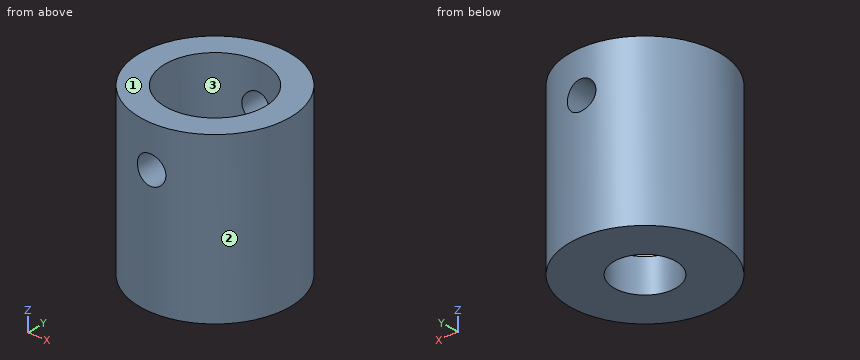
```python
from build123d import *

# Parameters (mm, degrees)
SKETCH1_R               = 58
SKETCH1_R_2             = 24
BOSS_EXTRUDE1_DEPTH     = 128
SKETCH2_R               = 38
CUT_EXTRUDE1_DEPTH      = 102
CUT_EXTRUDE2_DEPTH      = 153.026313512
CUT_EXTRUDE2_DEPTH_BACK = 153.026313512
SKETCH3_R               = 11
SKETCH6_R               = 38.5
CUT_EXTRUDE3_DEPTH      = 68
SKETCH7_R               = 40
CUT_EXTRUDE4_DEPTH      = 4


with BuildPart() as part:
    # Sketch1 → Boss-Extrude1 (new body)
    with BuildSketch(Plane.XY):
        Circle(SKETCH1_R)
        Circle(SKETCH1_R_2, mode=Mode.SUBTRACT)
    extrude(amount=BOSS_EXTRUDE1_DEPTH)

    # Sketch2 → Cut-Extrude1 (cut)
    with BuildSketch(Plane.XY.offset(128)):
        Circle(SKETCH2_R)
    extrude(amount=-CUT_EXTRUDE1_DEPTH, mode=Mode.SUBTRACT)

    # Sketch3 → Cut-Extrude2 (cut, two sides: drawn at the far end of the back side and taken through both)
    with BuildSketch(Plane(origin=(0, 0, 0), x_dir=(1, 0, 0), z_dir=(0, 1, 0)).offset(-CUT_EXTRUDE2_DEPTH_BACK)):
        with Locations(Location((0, -96, 0), (0, 0, 270))):
            Circle(SKETCH3_R)
    extrude(amount=CUT_EXTRUDE2_DEPTH + CUT_EXTRUDE2_DEPTH_BACK, mode=Mode.SUBTRACT)

    # Sketch6 → Cut-Extrude3 (cut)
    with BuildSketch(Plane.XY.offset(128)):
        Circle(SKETCH6_R)
    extrude(amount=-CUT_EXTRUDE3_DEPTH, mode=Mode.SUBTRACT)

    # Sketch7 → Cut-Extrude4 (cut)
    with BuildSketch(Plane.XY.offset(60)):
        Circle(SKETCH7_R)
    extrude(amount=CUT_EXTRUDE4_DEPTH, mode=Mode.SUBTRACT)


solid = part.part
```
For this review, take the finished solid that the model builds, in its own axes (mm). Face numbers are marked on the shaded views. Coordinates: 2 decimals unless noted, no trailing zeros. Loops run counter-clockwise (first coordinate to the right, second up) from the corner with the lowest first, then second, coordinate; pieces in that order, holes last.
1. For line 1 (Z direction, x = 0, y = -50.5); line 2 (Y direction, x = 0, z = 63.1); line 3 (Y direction, x = 0, z = 7), list the stretches that pass through material, from the lowest coordinate up.
2. Mouldability with a two-part tool opening along Y and no side actions: class the marked faces 1, 2 and 3 as +Y half, -Y half, draft (parallel to the pull), parting line (faces both ways), or undercut.
3. Add section A-A, the plane y = 0. Give the boundary of the cut face in (x, z), then the cut area to 3 significant figures.
4. Add section B-B, the plane x = 0. Give the boundary of the cut face in (y, z).
5. Add section C-C, the plane z = 96. Give the boundary of the cut face in (x, y).
6. Insertion check: P1, Ø1.5, axis at x = 30.5, y = 15, coming from the +Z side; P2, Ø10, axis at y = 38.5, z = 41, coming from the -X side; P3, Ø10, axis at y = -22.5, z = 81, coming from the -X side. Each pin has a flat end and moves straight along its axis. Give the tip position at first contact, or say it passes through.
7. Add section D-D, the plane x = -19.5. Give the boundary of the cut face in (y, z), then the cut area to 3 significant figures.
Result:
1. line 1: z = 0 to 85, 107 to 128
1. line 2: y = -58 to -40, 40 to 58
1. line 3: y = -58 to -24, 24 to 58
2. face 1: draft
2. face 2: parting line
2. face 3: undercut
3. outline: (-58, 0) - (-24, 0) - (-24, 26) - (-38, 26) - (-38, 60) - (-40, 60) - (-40, 64) - (-38.5, 64) - (-38.5, 128) - (-58, 128) - close; (24, 0) - (58, 0) - (58, 128) - (38.5, 128) - (38.5, 64) - (40, 64) - (40, 60) - (38, 60) - (38, 26) - (24, 26) - close
3. area: 5,770 mm2
4. outline: (-58, 0) - (-24, 0) - (-24, 26) - (-38, 26) - (-38, 60) - (-40, 60) - (-40, 64) - (-38.5, 64) - (-38.5, 85) - (-58, 85) - close; (-58, 107) - (-38.5, 107) - (-38.5, 128) - (-58, 128) - close; (24, 0) - (58, 0) - (58, 85) - (38.5, 85) - (38.5, 64) - (40, 64) - (40, 60) - (38, 60) - (38, 26) - (24, 26) - close; (38.5, 107) - (58, 107) - (58, 128) - (38.5, 128) - close
5. outline: (-11, -56.95) - (-11, -36.9) arc R38.5 cw to (-11, 36.9) - (-11, 56.95) arc R58 ccw to start; (11, -56.95) arc R58 ccw to (11, 56.95) - (11, 36.9) arc R38.5 cw to (11, -36.9) - close
6. P1: stops at z = 26
6. P2: stops at x = -47.35
6. P3: stops at x = -55.3
7. outline: (-54.62, 0) - (-13.99, 0) - (-13.99, 26) - (-32.62, 26) - (-32.62, 60) - (-34.92, 60) - (-34.92, 64) - (-33.2, 64) - (-33.2, 128) - (-54.62, 128) - close; (13.99, 0) - (54.62, 0) - (54.62, 128) - (33.2, 128) - (33.2, 64) - (34.92, 64) - (34.92, 60) - (32.62, 60) - (32.62, 26) - (13.99, 26) - close
7. area: 6,510 mm2
